```python
from build123d import *

# Parameters (mm, degrees)
SKETCH1_W             = 80
SKETCH1_H             = 20
BOSS_EXTRUDE1_DEPTH   = 10
SKETCH3_W             = 70
SKETCH3_H             = 10
CUT_EXTRUDE1_DEPTH    = 43.426406871
M4_TAPPED_HOLE2_D     = 3.3
M4_TAPPED_HOLE2_DEPTH = 10.1
M4_TAPPED_HOLE2_TIP   = 0.991420021
CHAMFER1_SIZE         = 1
M4_TAPPED_HOLE1_D     = 3.3
M4_TAPPED_HOLE1_DEPTH = 10.1
M4_TAPPED_HOLE1_TIP   = 0.991420021


with BuildPart() as part:
    # Sketch1 → Boss-Extrude1 (new body)
    with BuildSketch(Plane(origin=(0, 0, 0), x_dir=(0, 0, -1), z_dir=(1, 0, 0))):
        Rectangle(SKETCH1_W, SKETCH1_H)
    extrude(amount=BOSS_EXTRUDE1_DEPTH)

    # Sketch3 → Cut-Extrude1 (cut, through all)
    with BuildSketch(Plane.ZY):
        with Locations((-5, -5)):
            Rectangle(SKETCH3_W, SKETCH3_H)
    extrude(amount=-CUT_EXTRUDE1_DEPTH, mode=Mode.SUBTRACT)

    # M4 Tapped Hole2
    with Locations(Plane(origin=(0, 0, 30), x_dir=(-1, 0, 0), z_dir=(0, 0, -1))):
        with Locations((-5, -5)):
            Hole(M4_TAPPED_HOLE2_D / 2, depth=M4_TAPPED_HOLE2_DEPTH)
            with Locations((0, 0, -(M4_TAPPED_HOLE2_DEPTH + M4_TAPPED_HOLE2_TIP / 2))):  # 118° drill point
                Cone(0, M4_TAPPED_HOLE2_D / 2, M4_TAPPED_HOLE2_TIP, mode=Mode.SUBTRACT)

    # Chamfer1
    chamfer1_edges = [part.edges().sort_by_distance(p)[0] for p in [
        (0, 5, -40),
        (10, 5, -40),
        (10, -10, 35),
        (0, -10, 35),
    ]]
    chamfer(chamfer1_edges, length=CHAMFER1_SIZE)

    # M4 Tapped Hole1
    with Locations(Plane(origin=(0, 10, 0), x_dir=(1, 0, 0), z_dir=(0, 1, 0))):
        with Locations((5, 25), (5, -20)):
            Hole(M4_TAPPED_HOLE1_D / 2, depth=M4_TAPPED_HOLE1_DEPTH)
            with Locations((0, 0, -(M4_TAPPED_HOLE1_DEPTH + M4_TAPPED_HOLE1_TIP / 2))):  # 118° drill point
                Cone(0, M4_TAPPED_HOLE1_D / 2, M4_TAPPED_HOLE1_TIP, mode=Mode.SUBTRACT)


solid = part.part
```
Source: CAD feature listing. Evaluate the final solid. Frame: model axes, mm. A direction names the side the tool comes from. Give positions to 0.01 mm unless a question says otherwise; leave off trailing zeros. Loops run counter-clockwise (first coordinate to the right, second up) from the corner with the lowest first, then second, coordinate; pieces in that order, holes last. Notation, with made-up numbers: (15, -18.75) -> (50, -18.75) arc R23 cw to (50, -3.75) -> close; hole circle Ø10 at (86.25, -3.5). An arc over 180 degrees is marked (long way). Use a Markdown table: item, result. Add a question column.
(1) Section query A-A (y = -5). Output: boundary loops of the cut face in (x, z), then the cut area to 3 significant figures.
(2) Ray query, line 1 (Z direction, x = 5, y = 8.25); line 2 (Y direction, x = 5, z = 34.75); line 3 (Z direction, x = 3.5, y = 9). Return the intervals inside material, ascending.
(3) Section query B-B (x = 5). Output: boundary loops of the cut face in (y, z).
(4) Pull-direction query (Z, two-part tool) for faces 3 (the face through (5, 5, -40)), 4 (the face through (0, 5, 1)), 5 (the face through (5.215, 4.93, 18.364)), 6 (the face through (5.215, 4.93, -26.636)); classes: +Z half, -Z half, draft (parallel to the pull), parting line (faces both ways), or undercut.
(5) Access query for faces 1 (the face through (5, -3, 30)), 2 (the face through (3.35, -4.93, 35.07)). Directions: +Z, -Z, +X, -X, +Y, -Y. A direction counts if a zero-diameter tool reaches every point of the face in a straight line with its end or side. Return the directions, or none.
(6) First-contact query: pin 1 Ø5 at (x, y) = (6, -4.5) entering from -Z. Flat tip, straight axial feed; report the tip coordinate or a pass-through.
(7) Section query D-D (y = 7). Output: boundary loops of the cut face in (x, z).
(8) Section query C-C (z = -25). Output: boundary loops of the cut face in (x, y), then the cut area to 3 significant figures.
Checked values:
| question | item | result |
|---|---|---|
| 1 | outline | (0, 30) -> (3.35, 30) -> (3.35, 40) -> (0, 40) -> close; (6.65, 30) -> (10, 30) -> (10, 40) -> (6.65, 40) -> close |
| 1 | area | 67.0 mm^2 |
| 2 | line 1 | -40 to -26.65, -23.35 to 18.35, 21.65 to 40 |
| 2 | line 2 | -10 to -6.65, -3.35 to 10 |
| 2 | line 3 | -40 to -25.69, -24.31 to 19.31, 20.69 to 40 |
| 3 | outline | (-10, 30) -> (-6.65, 30) -> (-6.65, 40) -> (-10, 40) -> close; (-3.35, 30) -> (0, 30) -> (0, 21.65) -> (10, 21.65) -> (10, 40) -> (-3.35, 40) -> close; (0, -40) -> (10, -40) -> (10, -26.65) -> (0, -26.65) -> close; (0, -23.35) -> (10, -23.35) -> (10, 18.35) -> (0, 18.35) -> close |
| 4 | face 3 | -Z half |
| 4 | face 4 | draft |
| 4 | face 5 | undercut |
| 4 | face 6 | undercut |
| 5 | face 1 | -Z, +X, -X, -Y |
| 5 | face 2 | +Z, -Z |
| 6 | pin 1 | z = 30 |
| 7 | outline | (0, -39) -> (1, -40) -> (9, -40) -> (10, -39) -> (10, 40) -> (0, 40) -> close; hole circle Ø3.3 at (5, -25); hole circle Ø3.3 at (5, 20) |
| 8 | outline | (0, 0) -> (3.35, 0) -> (3.35, 10) -> (0, 10) -> close; (6.65, 0) -> (10, 0) -> (10, 10) -> (6.65, 10) -> close |
| 8 | area | 67.0 mm^2 |
